```python
from build123d import *

# Parameters (mm, degrees)
BOSS_EXTRUDE1_DEPTH = 3


with BuildPart() as part:
    # Sketch1 → Boss-Extrude1 (new body)
    with BuildSketch(Plane.XY):
        Polygon((213.585362106, 213.495304552), (253.585362106, 213.495304552), (253.585362106, 175.495304552), (248.585362106, 170.495304552), (218.585362106, 170.495304552), (213.585362106, 175.495304552), align=None)
        with BuildLine():
            Line((229.085362106, 181.745304552), (229.085362106, 188.745304552))
            ThreePointArc((229.085362106, 188.745304552), (233.585362106, 193.245304552), (238.085362106, 188.745304552))
            Line((238.085362106, 188.745304552), (238.085362106, 181.745304552))
            ThreePointArc((238.085362106, 181.745304552), (233.585362106, 177.245304552), (229.085362106, 181.745304552))
        make_face(mode=Mode.SUBTRACT)
    extrude(amount=BOSS_EXTRUDE1_DEPTH)


solid = part.part
```
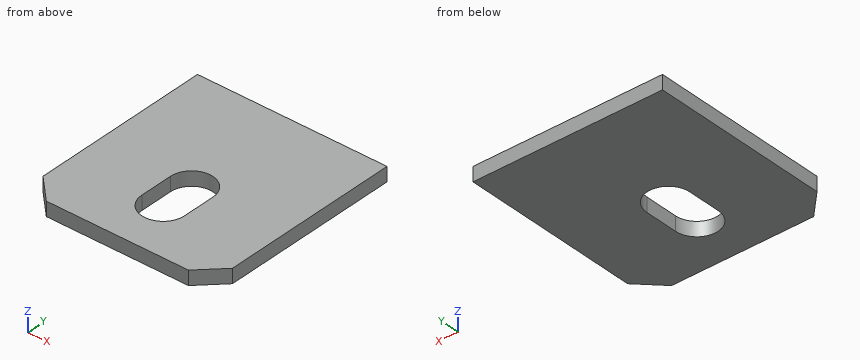
Check sheet for the modelled part. Datum: model origin and axes. Units: mm. Give positions to 0.01 mm unless a question says otherwise; leave off trailing zeros. Order: outer loops, then holes, each group sorted by start corner. A loop starts at its lowest first (then second) coordinate and runs counter-clockwise, first axis right, second up. Notation, with made-up numbers: M 84.5,45.25 L 138.5,45.25 A28 cw 138.5,65.25 Z; hole C 67,-30.75 d11. An arc over 180 degrees is marked long. Answer in a Markdown table with one row per item. Add a question column.
Q1. Sectioned sample at B-B, the plane y = 186.5. Record the boundary of the cut face in (x, z), and give its area (3 significant figures).
Q2. Thickness scan on L1, parallel to X at y = 183, z = 0.8; L2, parallel to Y at x = 233, z = 1.7; L3, parallel to X at y = 179, z = 2.55. Record the ranges inside material, lowest first.
Q3. Sectioned sample at A-A, the plane z = 1.9. Record the boundary of the cut face in (x, y), and give its area (3 significant figures).
Q4. Sectioned sample at C-C, the plane x = 230. Record the boundary of the cut face in (y, z), and give its area (3 significant figures).
Q5. Sectioned sample at D-D, the plane x = 250.5. Record the boundary of the cut face in (y, z), and give its area (3 significant figures).
Verdict:
| question | item | result |
|---|---|---|
| 1 | outline | M 213.59,0 L 229.09,0 L 229.09,3 L 213.59,3 Z; M 238.09,0 L 253.59,0 L 253.59,3 L 238.09,3 Z |
| 1 | area | 93.0 mm² |
| 2 | L1 | 213.59 to 229.09, 238.09 to 253.59 |
| 2 | L2 | 170.5 to 177.28, 193.21 to 213.5 |
| 2 | L3 | 213.59 to 230.02, 237.15 to 253.59 |
| 3 | outline | M 213.59,175.5 L 218.59,170.5 L 248.59,170.5 L 253.59,175.5 L 253.59,213.5 L 213.59,213.5 Z; hole M 229.09,181.75 A4.5 ccw 238.09,181.75 L 238.09,188.75 A4.5 ccw 229.09,188.75 Z |
| 3 | area | 1,570 mm² |
| 4 | outline | M 170.5,0 L 179.03,0 L 179.03,3 L 170.5,3 Z; M 191.46,0 L 213.5,0 L 213.5,3 L 191.46,3 Z |
| 4 | area | 91.7 mm² |
| 5 | outline | M 172.41,0 L 213.5,0 L 213.5,3 L 172.41,3 Z |
| 5 | area | 123 mm² |
